Could you check a few things on this model? Use its own coordinates, in mm. Give positions to 0.01 mm unless a question says otherwise; leave off trailing zeros. Order: outer loops, then holes, each group sorted by start corner. A loop starts at its lowest first (then second) coordinate and runs counter-clockwise, first axis right, second up. Notation, with made-up numbers: M 81,-29 L 119,-29 A7 cw 119,-21 Z; hole C 25.25,-37.75 d5. An arc over 180 degrees is marked long. Use a Markdown table: item, result. Add a question column.
Item 1: Suppose I cut it at C-C on y = 4.25. Write out the boundary of the cut face in (x, z).
Item 2: Suppose I cut it at A-A on z = 2.5. Write out the boundary of the cut face in (x, y).
Item 3: If I drill on L1, parallel to Z at x = -20, y = 12.25; L2, parallel to X at y = 13, z = 47.5; L3, parallel to Z at x = 0, y = 10.25, over which ranges is the centre line in solid material (lowest first)? Write a range as from..to.
Item 4: Suppose I cut it at B-B on x = -20. Write out the boundary of the cut face in (y, z).
Item 5: I'm going to push a flat-ended pin straight in: pin 1 Ø7.5 at (x, z) = (0, 47.5) entering from -Y. Where does the tip first touch, or does it pass through?
Item 6: If we mould it in two halves opening along Z, with no side actions, what happens to faces 1 (the face through (0, 12, -67.5)), 2 (the face through (0, 0, -1)), 3 (the face through (-16.868, 11.832, -0.372))? For each: released by +Z, released by -Z, zero draft, split by the parting line, or undercut.
Item 7: Suppose I cut it at D-D on z = 47.5. Write out the boundary of the cut face in (x, y), plus the area to 3 significant figures.
from build123d import *

# Parameters (mm, degrees)
SKETCH_1_W          = 70
SKETCH_1_H          = 135
EXTRUDE_1_DEPTH     = 24
HOLE_WIZARD_M10_1_D = 8.5


with BuildPart() as part:
    # 草图1 → 凸台-拉伸1 (new body)
    with BuildSketch(Plane(origin=(0, 0, 0), x_dir=(1, 0, 0), z_dir=(0, 1, 0))):
        Rectangle(SKETCH_1_W, SKETCH_1_H)
    extrude(amount=EXTRUDE_1_DEPTH)

    # M10 螺纹孔1 (through all)
    with Locations(Plane(origin=(0, 24, 0), x_dir=(1, 0, 0), z_dir=(0, 1, 0))):
        with Locations((-20, -2.5), (20, -2.5), (0, -47.5)):
            Hole(HOLE_WIZARD_M10_1_D / 2)


solid = part.part
Findings below:
| question | item | result |
|---|---|---|
| 1 | outline | M -35,-67.5 L 35,-67.5 L 35,67.5 L -35,67.5 Z; hole C -20,2.5 d8.5; hole C 0,47.5 d8.5; hole C 20,2.5 d8.5 |
| 2 | outline | M -35,0 L -24.25,0 L -24.25,24 L -35,24 Z; M -15.75,0 L 15.75,0 L 15.75,24 L -15.75,24 Z; M 24.25,0 L 35,0 L 35,24 L 24.25,24 Z |
| 3 | L1 | z = -67.5..-1.75, 6.75..67.5 |
| 3 | L2 | x = -35..-4.25, 4.25..35 |
| 3 | L3 | z = -67.5..43.25, 51.75..67.5 |
| 4 | outline | M 0,-67.5 L 24,-67.5 L 24,-1.75 L 0,-1.75 Z; M 0,6.75 L 24,6.75 L 24,67.5 L 0,67.5 Z |
| 5 | pin 1 | passes through |
| 6 | face 1 | released by -Z |
| 6 | face 2 | zero draft |
| 6 | face 3 | undercut |
| 7 | outline | M -35,0 L -4.25,0 L -4.25,24 L -35,24 Z; M 4.25,0 L 35,0 L 35,24 L 4.25,24 Z |
| 7 | area | 1,480 mm^2 |
